Check sheet for the modelled part. Datum: model origin and axes. Units: mm. A direction names the side the tool comes from. Coordinates: 2 decimals unless noted, no trailing zeros. Write each loop counter-clockwise with the first axis right and the second up, starting at its lowest first coordinate (ties: lowest second). Pieces come first, ordered by that corner, then holes. Notation, with made-up numbers: (18.5, -24.75) - (63.5, -24.75) arc R20 ccw to (63.5, -16.75) - close; hole circle Ø5 at (-33, -13.75). An arc over 180 degrees is marked (long way). Write each question's results on one line, items separated by ' | '.
from build123d import *

# Parameters (mm, degrees)
SKETCH1_W           = 210
SKETCH1_H           = 130
SKETCH1_R           = 3
BOSS_EXTRUDE1_DEPTH = 4
SKETCH2_W           = 48
SKETCH2_H           = 48
BOSS_EXTRUDE2_DEPTH = 11
SKETCH3_R           = 13.5
CUT_EXTRUDE1_DEPTH  = 11
SKETCH4_R           = 15.5
CUT_EXTRUDE2_DEPTH  = 11
SCALE_1_SCALE       = 1.875


with BuildPart() as part:
    # Sketch1 → Boss-Extrude1 (new body)
    with BuildSketch(Plane.XY):
        Rectangle(SKETCH1_W, SKETCH1_H)
        with Locations((97, 57)):
            Circle(SKETCH1_R, mode=Mode.SUBTRACT)
        with Locations((-97, 57)):
            Circle(SKETCH1_R, mode=Mode.SUBTRACT)
        with Locations((-97, -57)):
            Circle(SKETCH1_R, mode=Mode.SUBTRACT)
        with Locations((97, -57)):
            Circle(SKETCH1_R, mode=Mode.SUBTRACT)
    extrude(amount=BOSS_EXTRUDE1_DEPTH)

    # Sketch2 → Boss-Extrude2 (add)
    with BuildSketch(Plane(origin=(0, 0, 0), x_dir=(-1, 0, 0), z_dir=(0, 0, -1))):
        Rectangle(SKETCH2_W, SKETCH2_H)
    extrude(amount=BOSS_EXTRUDE2_DEPTH)

    # Sketch3 → Cut-Extrude1 (cut)
    with BuildSketch(Plane(origin=(0, 0, -11), x_dir=(-1, 0, 0), z_dir=(0, 0, -1))):
        Circle(SKETCH3_R)
    extrude(amount=-CUT_EXTRUDE1_DEPTH, mode=Mode.SUBTRACT)

    # Sketch4 → Cut-Extrude2 (cut)
    with BuildSketch(Plane(origin=(0, 0, 0), x_dir=(-1, 0, 0), z_dir=(0, 0, -1))):
        Circle(SKETCH4_R)
    extrude(amount=-CUT_EXTRUDE2_DEPTH, mode=Mode.SUBTRACT)


with BuildPart() as part_1:
    # Scale 1: scaled about (0, 0, 0.855180598)
    add(part.part.scale(SCALE_1_SCALE).moved(Location((0, 0, -0.748283023))))


solid = part_1.part
1. Go/stop test with flat-tipped pins: pin 1 (3 mm diameter, centred on x = -82.5, y = -72, fed in from -Z); pin 2 (12 mm diameter, centred on x = -34.5, z = -10.5, fed in from +Y); pin 3 (1 mm diameter, centred on x = 10.5, z = -10, fed in from -Y). Record where each tip stops, or that it passes through.
Values follow:
pin 1: stops at z = -0.75 | pin 2: stops at y = 45 | pin 3: stops at y = -45
2. Material ranges on L1, parallel to Y at x = 0, z = -8.75; L2, parallel to Y at x = 0, z = 4.5 (1 decimal); L3, parallel to Z at x = 58, y = 105, recorded low to high. Write a range as [from, to].
Values follow:
L1: y = [-45, -25.31], [25.31, 45] | L2: y = [-121.9, -29.1], [29.1, 121.9] | L3: z = [-0.75, 6.75]
3. Sectioned sample at A-A (x = 0). Record the cut outline in (y, z) (1 decimal), then the cut area to 3 significant figures.
Values follow:
outline: (-121.9, -0.7) - (-45, -0.7) - (-45, -21.4) - (-25.3, -21.4) - (-25.3, -0.7) - (-29.1, -0.7) - (-29.1, 6.8) - (-121.9, 6.8) - close; (25.3, -21.4) - (45, -21.4) - (45, -0.7) - (121.9, -0.7) - (121.9, 6.8) - (29.1, 6.8) - (29.1, -0.7) - (25.3, -0.7) - close | area: 2,200 mm^2
4. Sectioned sample at B-B (y = 0). Record the cut outline in (x, z) (1 decimal), then the cut area to 3 significant figures.
Values follow:
outline: (-196.9, -0.7) - (-45, -0.7) - (-45, -21.4) - (-25.3, -21.4) - (-25.3, -0.7) - (-29.1, -0.7) - (-29.1, 6.8) - (-196.9, 6.8) - close; (25.3, -21.4) - (45, -21.4) - (45, -0.7) - (196.9, -0.7) - (196.9, 6.8) - (29.1, 6.8) - (29.1, -0.7) - (25.3, -0.7) - close | area: 3,330 mm^2
5. Access from +Z, -Z, +X, -X, +Y, -Y to the whole of each face (thin tool, end or side, straight path). Record for faces 1 (the flat face through (1, 45, -11)), 2 (the flat face through (41, 2, 6.752)), 3 (the flat face through (1, -45, -11)), 4 (the cylindrical face through (23.063, -17.684, 2.949)), 5 (the flat face through (-45, -1, -11)).
Values follow:
face 1: -Z, +X, -X, +Y | face 2: +Z, +X, -X, +Y, -Y | face 3: -Z, +X, -X, -Y | face 4: +Z | face 5: -Z, -X, +Y, -Y
6. Sectioned sample at C-C (z = -11.5). Record the cut outline in (x, y) (1 decimal).
Values follow:
outline: (-45, -45) - (45, -45) - (45, 45) - (-45, 45) - close; hole circle Ø50.6 at (0, 0)
7. Draft check along X on faces 6 (the flat face through (45, -1, -11)), 7 (the flat face through (-3, 121.875, 3)), 8 (the cylindrical face through (-178.9, -102.1, 2.9)). Enter one of: pulls with the +X half, pulls with the -X half, needs draft (parallel to the pull), parting line crosses it, or undercut.
Values follow:
face 6: pulls with the +X half | face 7: needs draft | face 8: undercut
8. Sectioned sample at D-D (y = 35). Record the cut outline in (x, z) (3 decimals), then the cut area to 3 significant figures.
Values follow:
outline: (-196.875, -0.748) - (-45, -0.748) - (-45, -21.373) - (45, -21.373) - (45, -0.748) - (196.875, -0.748) - (196.875, 6.752) - (-196.875, 6.752) - close | area: 4,810 mm^2
